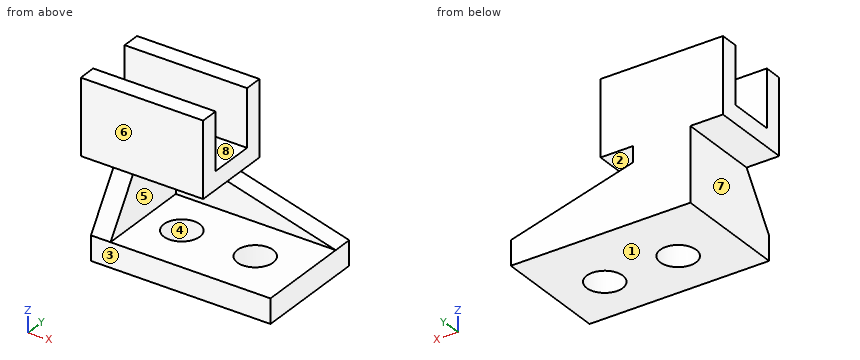
from build123d import *

# Parameters (mm, degrees)
BASE_PLATE_SKETCH_W         = 110
BASE_PLATE_SKETCH_H         = 70
BASE_PLATE_15MM_DEPTH       = 15
TRIANGULAR_WALL_12MM_DEPTH  = 12
WALL_EXTENSION_12MM_DEPTH   = 12
WEDGE_GUSSET_12MM_DEPTH     = 12
TOP_PROFILE_BOSS_11MM_DEPTH = 11
PROFILE_ARM_75MM_DEPTH      = 75
BLOCK_ARM_SKETCH_W          = 24
BLOCK_ARM_SKETCH_H          = 11
BLOCK_ARM_75MM_DEPTH        = 75
HOLE_CIRCLES_2X_22_SKETCH_R = 11
HOLES_2X_22_DEPTH           = 15
UPPER_JAW_SKETCH_W          = 11
UPPER_JAW_SKETCH_H          = 11
UPPER_JAW_75MM_DEPTH        = 75
LOWER_JAW_SKETCH_W          = 11
LOWER_JAW_SKETCH_H          = 11
LOWER_JAW_75MM_DEPTH        = 75


with BuildPart() as part:
    # Base Plate Sketch → Base Plate 15mm (new body)
    with BuildSketch(Plane.XY):
        with Locations((55, 35)):
            Rectangle(BASE_PLATE_SKETCH_W, BASE_PLATE_SKETCH_H)
    extrude(amount=BASE_PLATE_15MM_DEPTH)

    # Triangular Wall Sketch → Triangular Wall 12mm (add)
    with BuildSketch(Plane(origin=(0, 70, 0), x_dir=(1, 0, 0), z_dir=(0, 1, 0))):
        Polygon((0, -15), (0, -45), (110, -15), align=None)
    extrude(amount=-TRIANGULAR_WALL_12MM_DEPTH)

    # Wall Extension Sketch → Wall Extension 12mm (add)
    with BuildSketch(Plane.ZY):
        Polygon((45, 58), (45, 20), (15, 0), (15, 58), align=None)
    extrude(amount=-WALL_EXTENSION_12MM_DEPTH)

    # Wedge Gusset Sketch → Wedge Gusset 12mm (add)
    with BuildSketch(Plane(origin=(0, 70, 0), x_dir=(1, 0, 0), z_dir=(0, 1, 0))):
        Polygon((0, -45), (35, -45), (35, -35.454545455), align=None)
    extrude(amount=-WEDGE_GUSSET_12MM_DEPTH)

    # Top Profile Sketch → Top Profile Boss 11mm (add)
    with BuildSketch(Plane(origin=(0, 70, 0), x_dir=(1, 0, 0), z_dir=(0, 1, 0))):
        Polygon((17.5, -45), (55, -45), (55, -56), (-20, -56), (-20, -45), align=None)
    extrude(amount=-TOP_PROFILE_BOSS_11MM_DEPTH)

    # Profile Arm Sketch → Profile Arm 75mm (add)
    with BuildSketch(Plane(origin=(55, 0, 0), x_dir=(0, 0, -1), z_dir=(1, 0, 0))):
        Polygon((-45, 59), (-45, 31), (-45, 20), (-80, 20), (-80, 31), (-56, 31), (-56, 59), align=None)
    extrude(amount=-PROFILE_ARM_75MM_DEPTH)

    # Block Arm Sketch → Block Arm 75mm (add)
    with BuildSketch(Plane(origin=(55, 0, 0), x_dir=(0, 0, -1), z_dir=(1, 0, 0))):
        with Locations((-68, 64.5)):
            Rectangle(BLOCK_ARM_SKETCH_W, BLOCK_ARM_SKETCH_H)
    extrude(amount=-BLOCK_ARM_75MM_DEPTH)

    # Hole Circles 2xØ22 Sketch → Holes 2xØ22 (cut)
    with BuildSketch(Plane.XY.offset(15)):
        with Locations((80, 30)):
            Circle(HOLE_CIRCLES_2X_22_SKETCH_R)
        with Locations((35, 30)):
            Circle(HOLE_CIRCLES_2X_22_SKETCH_R)
    extrude(amount=-HOLES_2X_22_DEPTH, mode=Mode.SUBTRACT)

    # Upper Jaw Sketch → Upper Jaw 75mm (add)
    with BuildSketch(Plane(origin=(55, 0, 0), x_dir=(0, 0, -1), z_dir=(1, 0, 0))):
        with Locations((-85.5, 64.5)):
            Rectangle(UPPER_JAW_SKETCH_W, UPPER_JAW_SKETCH_H)
    extrude(amount=-UPPER_JAW_75MM_DEPTH)

    # Lower Jaw Sketch → Lower Jaw 75mm (add)
    with BuildSketch(Plane(origin=(55, 0, 0), x_dir=(0, 0, -1), z_dir=(1, 0, 0))):
        with Locations((-85.5, 25.5)):
            Rectangle(LOWER_JAW_SKETCH_W, LOWER_JAW_SKETCH_H)
    extrude(amount=-LOWER_JAW_75MM_DEPTH)


solid = part.part
Check sheet for the modelled part. Datum: model origin and axes. Units: mm. Face numbers are marked on the shaded views. A direction names the side the tool comes from. Give positions to 0.01 mm unless a question says otherwise; leave off trailing zeros. Write each loop counter-clockwise with the first axis right and the second up, starting at its lowest first coordinate (ties: lowest second). Pieces come first, ordered by that corner, then holes. Notation, with made-up numbers: (53.5, 12) -> (81.5, 12) arc R23 cw to (81.5, 51) -> close; hole circle Ø3 at (-25, 5.25). An arc over 180 degrees is marked (long way). Use one line per item in the form item = value. Start each with the question number.
1. Thickness scan on line 1 along Y through (x, z) = (35, 11); line 2 along Z through (x, y) = (17, 36); line 3 along Y through (x, z) = (-4.5, 61.5). Record the ranges inside material, lowest first. Write a range as from..to.
2. Go/stop test with flat-tipped pins: P1, Ø14, axis at x = 14.5, y = 38.5, coming from the +Z side; P2, Ø10.5, axis at x = 16.5, z = 70, coming from the -Y side; P3, Ø1.5, axis at y = 50, z = 53, coming from the +X side. Record where each tip stops, or that it passes through.
3. Access from +Z, -Z, +X, -X, +Y, -Y to the whole of each face (thin tool, end or side, straight path). Record for the marked faces 4, 5, 6, 7 and 8.
4. Section check C-C (y = 49.5). Record the cut outline in (x, z), and give its area (4 significant figures).
5. Section check A-A (z = 61.5). Record the cut outline in (x, y), and give its area (3 significant figures).
6. Mould release check, pull along Z, two halves, no side actions. Record for the marked faces 1, 2 and 3: pulls with the +Z half, pulls with the -Z half, needs draft (parallel to the pull), parting line crosses it, or undercut.
7. Section check B-B (x = 49). Record the cut outline in (y, z).
8. Section check D-D (y = 27). Record the cut outline in (x, z), and give its area (3 significant figures).
Conclusion:
q1.line_1 = 0..19, 41..70
q1.line_2 = 0..15, 45..56
q1.line_3 = 20..31, 59..70
q2.P1 = 56
q2.P2 = 20
q2.P3 = 55
q3.face_4 = -Z
q3.face_5 = +X, -Y
q3.face_6 = +Z, +X, -X, -Y
q3.face_7 = -Z, -X, +Y, -Y
q3.face_8 = +Z, +X, -X
q4.outline = (-20, 45) -> (0, 45) -> (0, 0) -> (110, 0) -> (110, 15) -> (12, 15) -> (12, 45) -> (55, 45) -> (55, 56) -> (-20, 56) -> close
q4.area = 2,835 mm²
q5.outline = (-20, 20) -> (55, 20) -> (55, 31) -> (-20, 31) -> close; (-20, 59) -> (55, 59) -> (55, 70) -> (-20, 70) -> close
q5.area = 1,650 mm²
q6.face_1 = pulls with the -Z half
q6.face_2 = undercut
q6.face_3 = needs draft
q7.outline = (0, 0) -> (70, 0) -> (70, 31.64) -> (58, 31.64) -> (58, 15) -> (0, 15) -> close; (20, 45) -> (70, 45) -> (70, 91) -> (59, 91) -> (59, 56) -> (31, 56) -> (31, 91) -> (20, 91) -> close
q8.outline = (-20, 45) -> (0, 45) -> (0, 0) -> (24.42, 0) -> (24.42, 15) -> (12, 15) -> (12, 45) -> (55, 45) -> (55, 91) -> (-20, 91) -> close; (45.58, 0) -> (69.42, 0) -> (69.42, 15) -> (45.58, 15) -> close; (90.58, 0) -> (110, 0) -> (110, 15) -> (90.58, 15) -> close
q8.area = 4,830 mm²
